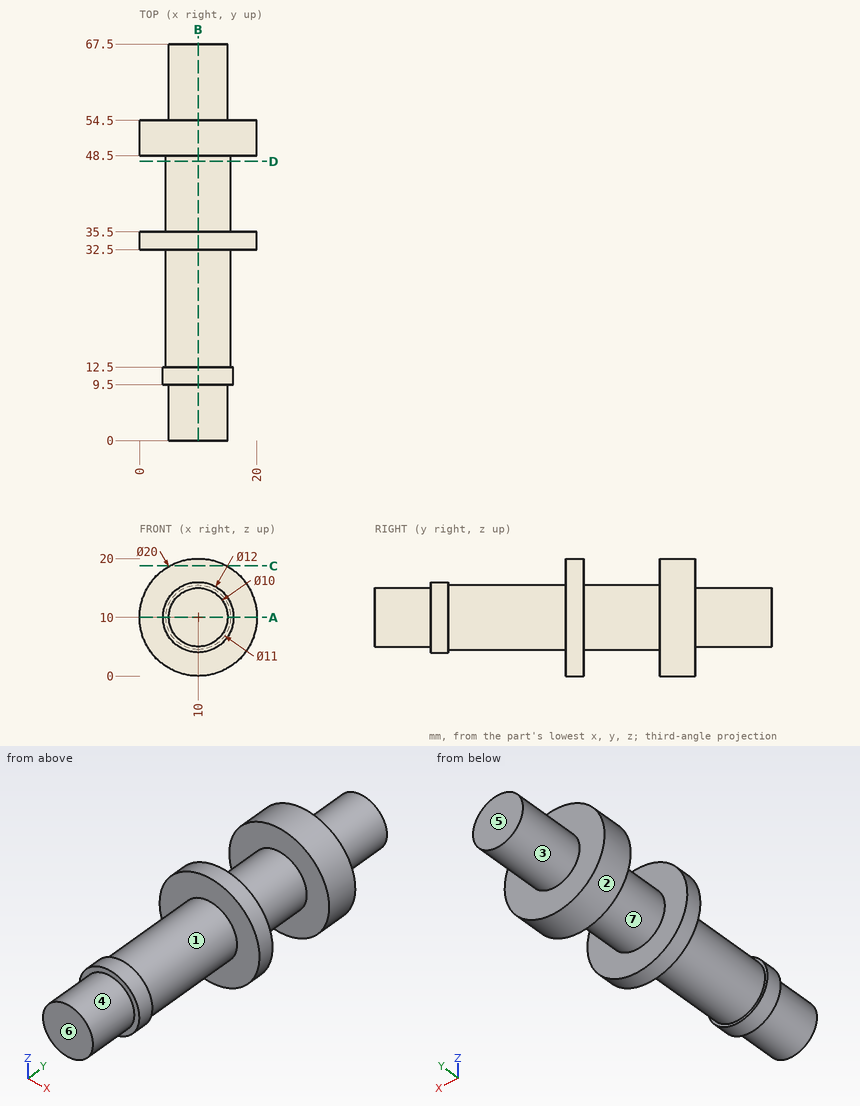
The drawing under review shows one solid part. Ordinate dimensions are in mm from its lowest x, y, z. A direction names the side the tool comes from. Give positions to 0.01 mm unless a question says otherwise; leave off trailing zeros. Order: outer loops, then holes, each group sorted by start corner. A loop starts at its lowest first (then second) coordinate and runs counter-clockwise, first axis right, second up. Notation, with made-up numbers: (21.5, 72.25) -> (63.5, 72.25) arc R25 cw to (63.5, 93.25) -> close; hole circle Ø1 at (65.25, -39.5). An arc over 180 degrees is marked (long way). Write item = value, one per line. Start each with the question number.
(1) We need section B-B on x = 10. Write out the cut boundary in (y, z), plus the area to 3 significant figures.
(2) We need section A-A on z = 10. Write out the cut boundary in (x, y), plus the area to 3 significant figures.
(3) For the marked faces 1, 2, 3 and 4, list the 3-axis set-ups (+Z, -Z, +X, -X, +Y, -Y) from which the entire face can be reached by the end or side of a thin tool; tool diameter is ignored.
(4) To check wall thickness, follow line 1 along Y through (x, z) = (1.25, 14.25); line 2 along Y through (x, z) = (4.5, 12.25); line 3 along Z through (x, y) = (10, 7). State the ranges of each line that lie inside material, in increasing order.
(5) For pin 1 (1 mm diameter, centred on x = 10, y = 43, fed in from -Z); pin 2 (3 mm diameter, centred on x = 17.5, z = 8.5, fed in from +Y); pin 3 (1 mm diameter, centred on x = 9, y = 57, fed in from -Z), all flat-tipped, find the tip position at first contact; note any pin that passes through.
(6) We need section C-C on z = 18.75. Write out the cut boundary in (x, y).
(7) Mouldability with a two-part tool opening along Y and no side actions: class the marked faces 5, 6 and 7 as +Y half, -Y half, draft (parallel to the pull), parting line (faces both ways), or undercut.
(8) We need section D-D on y = 47.5. Write out the cut boundary in (x, z).
Numbers:
q1.outline = (0, 5) -> (9.5, 5) -> (9.5, 4) -> (12.5, 4) -> (12.5, 4.5) -> (32.5, 4.5) -> (32.5, 0) -> (35.5, 0) -> (35.5, 4.5) -> (48.5, 4.5) -> (48.5, 0) -> (54.5, 0) -> (54.5, 5) -> (67.5, 5) -> (67.5, 15) -> (54.5, 15) -> (54.5, 20) -> (48.5, 20) -> (48.5, 15.5) -> (35.5, 15.5) -> (35.5, 20) -> (32.5, 20) -> (32.5, 15.5) -> (12.5, 15.5) -> (12.5, 16) -> (9.5, 16) -> (9.5, 15) -> (0, 15) -> close
q1.area = 804 mm^2
q2.outline = (0, 32.5) -> (4.5, 32.5) -> (4.5, 12.5) -> (4, 12.5) -> (4, 9.5) -> (5, 9.5) -> (5, 0) -> (15, 0) -> (15, 9.5) -> (16, 9.5) -> (16, 12.5) -> (15.5, 12.5) -> (15.5, 32.5) -> (20, 32.5) -> (20, 35.5) -> (15.5, 35.5) -> (15.5, 48.5) -> (20, 48.5) -> (20, 54.5) -> (15, 54.5) -> (15, 67.5) -> (5, 67.5) -> (5, 54.5) -> (0, 54.5) -> (0, 48.5) -> (4.5, 48.5) -> (4.5, 35.5) -> (0, 35.5) -> close
q2.area = 804 mm^2
q3.face_1 = none
q3.face_2 = +Y, -Y
q3.face_3 = +Y
q3.face_4 = -Y
q4.line_1 = 32.5 to 35.5, 48.5 to 54.5
q4.line_2 = 9.5 to 12.5, 32.5 to 35.5, 48.5 to 54.5
q4.line_3 = 5 to 15
q5.pin_1 = 4.5
q5.pin_2 = 54.5
q5.pin_3 = 5.03
q6.outline = (5.16, 32.5) -> (14.84, 32.5) -> (14.84, 35.5) -> (5.16, 35.5) -> close; (5.16, 48.5) -> (14.84, 48.5) -> (14.84, 54.5) -> (5.16, 54.5) -> close
q7.face_5 = +Y half
q7.face_6 = -Y half
q7.face_7 = undercut
q8.outline = circle Ø11 at (10, 10)
